from build123d import *

# Parameters (mm, degrees)
BASE_PLATE_DEPTH  = 10
SLOT_CUT_DEPTH    = 10
LUG_1_DEPTH       = 10
LUG_START         = -10
LUG_2_DEPTH       = 10
PIN_HOLE_SKETCH_R = 12.5
PIN_HOLE_25_DEPTH = 50


with BuildPart() as part:
    # Base Plate Sketch → Base Plate (new body)
    with BuildSketch(Plane.XY):
        with BuildLine():
            Line((95, 25), (0, 25))
            Line((0, 25), (0, -25))
            Line((0, -25), (95, -25))
            ThreePointArc((95, -25), (120, 0), (95, 25))
        make_face()
    extrude(amount=BASE_PLATE_DEPTH)

    # Slot Sketch → Slot Cut (cut)
    with BuildSketch(Plane.XY.offset(10)):
        with BuildLine():
            Line((65, 10), (95, 10))
            ThreePointArc((95, 10), (105, 0), (95, -10))
            Line((95, -10), (65, -10))
            ThreePointArc((65, -10), (55, 0), (65, 10))
        make_face()
    extrude(amount=-SLOT_CUT_DEPTH, mode=Mode.SUBTRACT)

    # Lug 1 Sketch → Lug 1 (add)
    with BuildSketch(Plane.XZ.offset(25)):
        with BuildLine():
            Line((0, 10), (0, 30))
            ThreePointArc((0, 30), (20, 50), (40, 30))
            Line((40, 30), (40, 20))
            ThreePointArc((40, 20), (42.928932188, 12.928932188), (50, 10))
            Line((50, 10), (0, 10))
        make_face()
    extrude(amount=-LUG_1_DEPTH)

    # Lug 2 Sketch → Lug 2 (add)
    with BuildSketch(Plane(origin=(0, 25, 0), x_dir=(1, 0, 0), z_dir=(0, 1, 0)).offset(LUG_START)):
        with BuildLine():
            Line((0, -30), (0, -10))
            Line((0, -10), (50, -10))
            ThreePointArc((50, -10), (42.928932188, -12.928932188), (40, -20))
            Line((40, -20), (40, -30))
            ThreePointArc((40, -30), (20, -50), (0, -30))
        make_face()
    extrude(amount=LUG_2_DEPTH)

    # Pin Hole Sketch → Pin Hole Ø25 (cut)
    with BuildSketch(Plane.XZ.offset(25)):
        with Locations(Location((20, 30, 0), (0, 0, 270))):
            Circle(PIN_HOLE_SKETCH_R)
    extrude(amount=-PIN_HOLE_25_DEPTH, mode=Mode.SUBTRACT)


solid = part.part
Geometry check sheet. Reference: the model listing, model coordinates, mm. A direction names the side the tool comes from. Give positions to 0.01 mm unless a question says otherwise; leave off trailing zeros. Order: outer loops, then holes, each group sorted by start corner. A loop starts at its lowest first (then second) coordinate and runs counter-clockwise, first axis right, second up.
1) Cross-section at A-A (x = 70). Record the boundary of the cut face in (y, z).
Results are:
outline: (-25, 0) - (-10, 0) - (-10, 10) - (-25, 10) - close; (10, 0) - (25, 0) - (25, 10) - (10, 10) - close
2) Draft check along Y on faces 6 (the cylindrical face through (105, 0, 5)), 7 (the flat face through (40, -20, 25)), 8 (the flat face through (38, 25, 14)). Enter one of: released by +Y, released by -Y, zero draft, split by the parting line, or undercut.
Results are:
face 6: undercut
face 7: zero draft
face 8: released by +Y
3) Tool access check on faces 1 (the flat face through (20, 15, 16)), 2 (the cylindrical face through (20.55, -20.07, 42.488)), 3 (the cylindrical face through (55, 0, 5)), 4 (the flat face through (40, 20, 25)), 5 (the flat face through (59, 11, 10)). Record the directions out of +Z, -Z, +X, -X, +Y, -Y that give a thin tool (end or side, any length) a straight path to the whole face; none if there is none.
Results are:
face 1: +Z, +X, -X
face 2: +Y, -Y
face 3: +Z, -Z
face 4: +Z, +X, +Y, -Y
face 5: +Z, +X
4) Cross-section at D-D (x = 20). Record the boundary of the cut face in (y, z).
Results are:
outline: (-25, 0) - (25, 0) - (25, 17.5) - (15, 17.5) - (15, 10) - (-15, 10) - (-15, 17.5) - (-25, 17.5) - close; (-25, 42.5) - (-15, 42.5) - (-15, 50) - (-25, 50) - close; (15, 42.5) - (25, 42.5) - (25, 50) - (15, 50) - close
5) Cross-section at B-B (y = 0). Record the boundary of the cut face in (x, z), then the cut area to 3 significant figures.
Results are:
outline: (0, 0) - (55, 0) - (55, 10) - (0, 10) - close; (105, 0) - (120, 0) - (120, 10) - (105, 10) - close
area: 700 mm2
6) Material ranges on probe 1 along X at (y, z) = (-21.75, 30); probe 2 along Y at (x, z) = (12.5, 11); probe 3 along Y at (x, z) = (76, 9.5), recorded low to high.
Results are:
probe 1: x = 0 to 7.5, 32.5 to 40
probe 2: y = -25 to -15, 15 to 25
probe 3: y = -25 to -10, 10 to 25
7) Gauge pin test, flat ends, axial feed: pin 1 (11 mm diameter, centred on y = -21.5, z = 27, fed in from +X); pin 2 (2 mm diameter, centred on x = 73, y = 12.5, fed in from +Z); pin 3 (15 mm diameter, centred on x = 79, y = 1.5, fed in from +Z). Record the tip position at first contact, or that the pin passes through.
Results are:
pin 1: stops at x = 40
pin 2: stops at z = 10
pin 3: passes through
8) Cross-section at C-C (z = 4). Record the boundary of the cut face in (x, y), then the cut area to 3 significant figures.
Results are:
outline: (0, -25) - (95, -25) arc R25 ccw to (95, 25) - (0, 25) - close; hole (65, -10) - (95, -10) arc R10 ccw to (95, 10) - (65, 10) arc R10 ccw to start
area: 4,820 mm2
